Read the model definition and answer for the solid it produces. Units are mm, in the model's axes. A direction names the side the tool comes from. Give positions to 0.01 mm unless a question says otherwise; leave off trailing zeros. Write each loop counter-clockwise with the first axis right and the second up, starting at its lowest first coordinate (ties: lowest second). Pieces come first, ordered by that corner, then holes. Notation, with made-up numbers: (-0.75, 35.25) -> (43.25, 35.25) arc R16 cw to (43.25, 45.25) -> close; hole circle Ø9 at (-23, 47). An arc over 180 degrees is marked (long way). Answer as CSV lines item,"result". Start each with the question number.
1. The part is cut by section A-A, the plane z = 71.5. Determine the outline of the cut face in (x, y), and give its area (3 significant figures).
2. The part is cut by section C-C, the plane x = 71.5. Determine the outline of the cut face in (y, z).
3. Find the intervals of material crossed by line 1 (Y direction, x = 101.5, z = 26); line 2 (Y direction, x = 55.5, z = 84); line 3 (Y direction, x = 45, z = 17.5), in increasing order.
4. For a pull along X with two mould halves and no side action, classify faces 6 (the flat face through (14, 30, 49)), 7 (the cylindrical face through (51.17, 247.47, 50.7)), 8 (the flat face through (27.5, 44, 49)) as pulls with the +X half, pulls with the -X half, needs draft (parallel to the pull), parting line crosses it, or undercut.
5. A tool of negligible diameter and unlimited length cuts with its end or side. For faces 1 (the flat face through (115, 15, 49)), 2 (the flat face through (57, 138, 100)), 3 (the flat face through (58, 118, 30)), 4 (the flat face through (11, 62, 49)), 5 (the flat face through (87.5, 43, 49)), from which of +Z, -Z, +X, -X, +Y, -Y can it reach the whole face along a straight path? Write none if from no direction.
6. The part is cut by section D-D, the plane z = 90. Determine the outline of the cut face in (x, y), and give its area (3 significant figures).
7. Given pin 1 (4 mm diameter, centred on y = 214.5, z = 70, fed in from -X); pin 2 (21.5 mm diameter, centred on y = 41, z = 53.5, fed in from +X); pin 3 (3 mm diameter, centred on y = 54, z = 80, fed in from -X), each flat-ended and moving along its own axis, determine where each tip first touches the part or whether it passes through.
8. The part is cut by section B-B, the plane x = 96.5. Determine the outline of the cut face in (y, z).
from build123d import *

# Parameters (mm, degrees)
SUPPORT_PROFILE_SKETCH_W         = 115
SUPPORT_PROFILE_SKETCH_H         = 30
SUPPORT_BODY_DEPTH               = 100
SIDE_MOUNTING_HOLES_SKETCH_R     = 15
SIDE_MOUNTING_HOLES_2X_DEPTH     = 324.8628221
OPEN_BEARING_SEAT_CUT_DEPTH      = 324.8628221
OPEN_BEARING_SEAT_CUT_DEPTH_BACK = 324.8628221


with BuildPart() as part:
    # Support Profile Sketch → Support Body (new body)
    with BuildSketch(Plane.XY):
        with BuildLine():
            Line((27.5, 57), (27.5, 30))
            Line((27.5, 30), (57.5, 30))
            Line((57.5, 30), (87.5, 30))
            Line((87.5, 30), (87.5, 57))
            ThreePointArc((87.5, 57), (88.964466094, 60.535533906), (92.5, 62))
            Line((92.5, 62), (115, 62))
            Line((115, 62), (115, 273))
            ThreePointArc((115, 273), (57.5, 285.765861395), (0, 273))
            Line((0, 273), (0, 62))
            Line((0, 62), (22.5, 62))
            ThreePointArc((22.5, 62), (26.035533906, 60.535533906), (27.5, 57))
        make_face()
        with Locations((57.5, 15)):
            Rectangle(SUPPORT_PROFILE_SKETCH_W, SUPPORT_PROFILE_SKETCH_H)
    extrude(amount=SUPPORT_BODY_DEPTH)

    # Side Mounting Holes Sketch → Side Mounting Holes 2x (cut, through all)
    with BuildSketch(Plane.XY.offset(100)):
        with Locations((53.126487568, 232.599577538)):
            Circle(SIDE_MOUNTING_HOLES_SKETCH_R)
        with Locations((53.126487568, 90.599577538)):
            Circle(SIDE_MOUNTING_HOLES_SKETCH_R)
    extrude(amount=-SIDE_MOUNTING_HOLES_2X_DEPTH, mode=Mode.SUBTRACT)

    # Bearing Seat Sketch → Open Bearing Seat Cut (cut, two sides: drawn at the far end of the back side and taken through both)
    with BuildSketch(Plane.ZY.offset(-OPEN_BEARING_SEAT_CUT_DEPTH_BACK)):
        with BuildLine():
            Line((-500.188374916, 118), (0, 118))
            Line((0, 118), (60, 118))
            ThreePointArc((60, 118), (79.41198533, 152.294805029), (60, 186.589610057))
            Line((60, 186.589610057), (0, 186.589610057))
            Line((0, 186.589610057), (0, 273))
            Line((0, 273), (100, 273))
            Line((100, 273), (100, 180.5))
            Line((100, 180.5), (108, 180.5))
            Line((108, 180.5), (108, 135.5))
            Line((108, 135.5), (100, 135.5))
            Line((100, 135.5), (100, 62))
            Line((100, 62), (100, -438.188374916))
            Line((100, -438.188374916), (779.965669758, 295.569302764))
            Line((779.965669758, 295.569302764), (179.777294842, 851.75767768))
            Line((179.777294842, 851.75767768), (-500.188374916, 118))
        make_face()
    extrude(amount=OPEN_BEARING_SEAT_CUT_DEPTH + OPEN_BEARING_SEAT_CUT_DEPTH_BACK, mode=Mode.SUBTRACT)


solid = part.part
Results found:
1,outline,"(0, 0) -> (115, 0) -> (115, 30) -> (87.5, 30) -> (87.5, 57) arc R5 cw to (92.5, 62) -> (115, 62) -> (115, 128.41) -> (0, 128.41) -> (0, 62) -> (22.5, 62) arc R5 cw to (27.5, 57) -> (27.5, 30) -> (0, 30) -> close; (0, 176.18) -> (115, 176.18) -> (115, 273) -> (0, 273) -> close; hole circle Ø30 at (53.13, 90.6); hole circle Ø30 at (53.13, 232.6)"
1,area,"22,700 mm²"
2,outline,"(0, 0) -> (118, 0) -> (118, 60) arc R40 cw to (186.59, 60) -> (186.59, 0) -> (273, 0) -> (273, 100) -> (0, 100) -> close"
3,line 1,"y = 0 to 30, 62 to 118, 186.59 to 273"
3,line 2,"y = 0 to 75.79, 105.41 to 217.79, 247.41 to 273"
3,line 3,"y = 0 to 77.99, 103.21 to 118, 186.59 to 219.99, 245.21 to 273"
4,face 6,"needs draft"
4,face 7,"undercut"
4,face 8,"pulls with the -X half"
5,face 1,"+Z, -Z, +X, +Y, -Y"
5,face 2,"+Z, +X, -X, +Y, -Y"
5,face 3,"-Z, +X, -X"
5,face 4,"+Z, -Z, -X"
5,face 5,"+Z, -Z, +X"
6,outline,"(0, 0) -> (115, 0) -> (115, 30) -> (87.5, 30) -> (87.5, 57) arc R5 cw to (92.5, 62) -> (115, 62) -> (115, 273) -> (0, 273) -> (0, 62) -> (22.5, 62) arc R5 cw to (27.5, 57) -> (27.5, 30) -> (0, 30) -> close; hole circle Ø30 at (53.13, 90.6); hole circle Ø30 at (53.13, 232.6)"
6,area,"28,200 mm²"
7,pin 1,"stops at x = 0"
7,pin 2,"stops at x = 87.5"
7,pin 3,"stops at x = 27.5"
8,outline,"(0, 0) -> (30, 0) -> (30, 100) -> (0, 100) -> close; (62, 0) -> (118, 0) -> (118, 60) arc R40 cw to (186.59, 60) -> (186.59, 0) -> (273, 0) -> (273, 100) -> (62, 100) -> close"
